Part model, mm, in its own coordinate system. Give positions to 0.01 mm unless a question says otherwise; leave off trailing zeros. Write each loop counter-clockwise with the first axis right and the second up, starting at its lowest first coordinate (ties: lowest second). Pieces come first, ordered by that corner, then holes.
from build123d import *

# Parameters (mm, degrees)
SKETCH1_W           = 205
SKETCH1_H           = 160
BOSS_EXTRUDE1_DEPTH = 10
SKETCH2_R           = 10.75
CUT_EXTRUDE1_DEPTH  = 131.408013557
M4_TAPPED_HOLE1_D   = 3.3
CHAMFER1_SIZE       = 2


with BuildPart() as part:
    # Sketch1 → Boss-Extrude1 (new body)
    with BuildSketch(Plane.XY):
        Rectangle(SKETCH1_W, SKETCH1_H)
    extrude(amount=BOSS_EXTRUDE1_DEPTH)

    # Sketch2 → Cut-Extrude1 (cut, through all)
    with BuildSketch(Plane.XY.offset(10)):
        with Locations((-78.5, -58)):
            Circle(SKETCH2_R)
        with Locations(Location((-78.5, 58, 0), (0, 0, 180))):
            Circle(SKETCH2_R)
        with Locations(Location((78.5, -58, 0), (0, 0, 180))):
            Circle(SKETCH2_R)
        with Locations((78.5, 58)):
            Circle(SKETCH2_R)
    extrude(amount=-CUT_EXTRUDE1_DEPTH, mode=Mode.SUBTRACT)

    # M4 Tapped Hole1 (through all)
    with Locations(Plane.XY.offset(10)):
        with Locations((-89.813708499, 69.313708499), (-67.186291501, 69.313708499), (-67.186291501, 46.686291501), (-89.813708499, 46.686291501), (67.186291501, 69.313708499), (89.813708499, 69.313708499), (67.186291501, 46.686291501), (89.813708499, 46.686291501), (-89.813708499, -46.686291501), (-67.186291501, -46.686291501), (-89.813708499, -69.313708499), (-67.186291501, -69.313708499), (67.186291501, -46.686291501), (89.813708499, -46.686291501), (67.186291501, -69.313708499), (89.813708499, -69.313708499)):
            Hole(M4_TAPPED_HOLE1_D / 2)

    # Chamfer1
    chamfer1_edges = [part.edges().sort_by_distance(p)[0] for p in [
        (102.5, -80, 5),
        (-102.5, -80, 5),
        (-102.5, 80, 5),
        (102.5, 80, 5),
    ]]
    chamfer(chamfer1_edges, length=CHAMFER1_SIZE)


solid = part.part
1) Saw through at B-B (x = 78.5). Write the cut outline in (y, z).
Check result:
outline: (-80, 0) - (-68.75, 0) - (-68.75, 10) - (-80, 10) - close; (-47.25, 0) - (47.25, 0) - (47.25, 10) - (-47.25, 10) - close; (68.75, 0) - (80, 0) - (80, 10) - (68.75, 10) - close
2) Saw through at C-C (z = 8.5). State how many separate pieces and enclosed holes the cut face has, and give its area (3 significant figures).
Check result:
separate pieces: 1
enclosed holes: 20
area: 31,200 mm2
3) Saw through at A-A (y = -58). Write the cut outline in (x, z).
Check result:
outline: (-102.5, 0) - (-89.25, 0) - (-89.25, 10) - (-102.5, 10) - close; (-67.75, 0) - (67.75, 0) - (67.75, 10) - (-67.75, 10) - close; (89.25, 0) - (102.5, 0) - (102.5, 10) - (89.25, 10) - close
4) Drill centre lines: L1, parallel to X at y = -47, z = 4.25; L2, parallel to Y at x = 78.5, z = 7.5; L3, parallel to X at y = -46.5, z = 8.5. Where is each one in solid material? Low to high.
Check result:
L1: x = -102.5 to -91.43, -88.19 to -68.81, -65.57 to 65.57, 68.81 to 88.19, 91.43 to 102.5
L2: y = -80 to -68.75, -47.25 to 47.25, 68.75 to 80
L3: x = -102.5 to -91.45, -88.17 to -68.83, -65.55 to 65.55, 68.83 to 88.17, 91.45 to 102.5
5) Mould opens along X. For faces 1 (the flat face through (-1, 1, 0)), 2 (the cylindrical face through (-73.54, -67.537, 5.07)), 3 (the flat face through (-102.5, -1, 5)) say: +X half, -X half, draft (parallel to the pull), parting line (faces both ways), or undercut.
Check result:
face 1: draft
face 2: undercut
face 3: -X half
6) Flat gauge pin, fed straight in: P1, Ø4.5, axis at x = 67.19, y = 69.31, coming from the +Z side. Where does the tip first touch, or does it go through?
Check result:
P1: stops at z = 10
